The model under review builds one solid part; all positions refer to its coordinate system, in mm. A direction names the side the tool comes from. Give positions to 0.01 mm unless a question says otherwise; leave off trailing zeros. Loops run counter-clockwise (first coordinate to the right, second up) from the corner with the lowest first, then second, coordinate; pieces in that order, holes last. Notation, with made-up numbers: (59, 31.5) -> (82, 31.5) arc R29 ccw to (82, 59.5) -> close; hole circle Ø10 at (-36.5, 3.25). An arc over 180 degrees is marked (long way). Write each question's results on one line, items separated by ' | '. Start each with the question number.
Q1. We need section C-C (z = -59). Write out the cut boundary in (x, y), plus the area to 3 significant figures.
Q2. Wall thickness on L1, parallel to X at y = 4.5, z = -12; L2, parallel to X at y = 8, z = -12; L3, parallel to X at y = 0.75, z = -70: over which ranges is each line inside the solid? List them lowest first. Write a range as [from, to].
Q3. We need section B-B (z = -68). Write out the cut boundary in (x, y).
Q4. We need section A-A (x = 75). Write out the cut boundary in (y, z).
Q5. Mouldability with a two-part tool opening along X and no side actions: class faces 3 (the face through (125, 6, -5)), 4 (the face through (8.242, 8.648, -73.495)), 5 (the face through (64, 12, -41)), 6 (the face through (0, 6, -39)) as released by +X, released by -X, zero draft, split by the parting line, or undercut.
Q6. Insertion check: pin 1 Ø12.5 at (x, z) = (18, -12) entering from +Y; pin 2 Ø5 at (x, z) = (8, -12) entering from +Y. Each pin has a flat end and moves straight along its axis. Give the tip position at first contact, or say it passes through.
Q7. Machinability: for faces 1 (the face through (18, 5.2, -8)), 2 (the face through (65.01, 6.08, -26.58)), which of the approach directions +Z, -Z, +X, -X, +Y, -Y give a long, thin tool a straight path to every point of the face, cutting with its end or side? Answer none if there is none.
Q8. We need section D-D (y = 8.5). Give the number of separate pieces and of enclosed holes in the cut face, plus the area to 3 significant figures.
from build123d import *

# Parameters (mm, degrees)
SKETCH1_W                                            = 130
SKETCH1_H                                            = 80
BOSS_EXTRUDE1_DEPTH                                  = 12
CHAMFER1_SIZE                                        = 10
CBORE_FOR_M6_HEXAGON_SOCKET_HEAD_CAP_SCR_D           = 6.6
CBORE_FOR_M6_HEXAGON_SOCKET_HEAD_CAP_SCR_CBORE_D     = 11
CBORE_FOR_M6_HEXAGON_SOCKET_HEAD_CAP_SCR_CBORE_DEPTH = 6.8
F_6_0MM_DOWEL_HOLE_1_D                               = 6
F_20_0MM_DOWEL_HOLE_1_D                              = 20
SKETCH17_R                                           = 2.5
CUT_EXTRUDE1_DEPTH                                   = 154.114336363


with BuildPart() as part:
    # Sketch1 → Boss-Extrude1 (new body)
    with BuildSketch(Plane(origin=(0, 0, 0), x_dir=(1, 0, 0), z_dir=(0, 1, 0))):
        with Locations((65, 40)):
            Rectangle(SKETCH1_W, SKETCH1_H)
    extrude(amount=BOSS_EXTRUDE1_DEPTH)

    # Chamfer1
    chamfer1_edges = [part.edges().sort_by_distance(p)[0] for p in [
        (130, 6, -80),
        (130, 6, 0),
    ]]
    chamfer(chamfer1_edges, length=CHAMFER1_SIZE)

    # CBORE for M6 Hexagon socket head cap screws1 (through all)
    with Locations(Plane(origin=(8, 12, -68), x_dir=(0, 0, 1), z_dir=(0, 1, 0))):
        with Locations((0, 0), (56, 10)):
            CounterBoreHole(CBORE_FOR_M6_HEXAGON_SOCKET_HEAD_CAP_SCR_D / 2, CBORE_FOR_M6_HEXAGON_SOCKET_HEAD_CAP_SCR_CBORE_D / 2, CBORE_FOR_M6_HEXAGON_SOCKET_HEAD_CAP_SCR_CBORE_DEPTH)

    # Ø6.0mm dowel hole 1 (through all)
    with Locations(Plane(origin=(18, 12, -68), x_dir=(0, 0, 1), z_dir=(0, 1, 0))):
        with Locations((0, 0), (56, -10)):
            Hole(F_6_0MM_DOWEL_HOLE_1_D / 2)

    # Ø20.0mm dowel hole 1 (through all)
    with Locations(Plane(origin=(0, 0, 0), x_dir=(-1, 0, 0), z_dir=(0, -1, 0))):
        with Locations((-75, 52.142135624), (-75, 26.142135624)):
            Hole(F_20_0MM_DOWEL_HOLE_1_D / 2)

    # Sketch17 → Cut-Extrude1 (cut, through all)
    with BuildSketch(Plane(origin=(0, 12, 0), x_dir=(1, 0, 0), z_dir=(0, 1, 0))):
        with Locations(Location((81, 6.142135624, 0), (0, 0, 270))):
            Circle(SKETCH17_R)
        with Locations(Location((69, 72.142135624, 0), (0, 0, 270))):
            Circle(SKETCH17_R)
    extrude(amount=-CUT_EXTRUDE1_DEPTH, mode=Mode.SUBTRACT)


solid = part.part
Output:
1) outline: (0, 0) -> (67.72, 0) -> (67.72, 12) -> (0, 12) -> close; (82.28, 0) -> (130, 0) -> (130, 12) -> (82.28, 12) -> close | area: 1,390 mm2
2) L1: [0, 5], [11, 14.7], [21.3, 130] | L2: [0, 5], [11, 12.5], [23.5, 130] | L3: [0, 5.38], [10.62, 15.76], [20.24, 67.71], [70.29, 130]
3) outline: (0, 0) -> (4.7, 0) -> (4.7, 5.2) -> (2.5, 5.2) -> (2.5, 12) -> (0, 12) -> close; (11.3, 0) -> (15, 0) -> (15, 12) -> (13.5, 12) -> (13.5, 5.2) -> (11.3, 5.2) -> close; (21, 0) -> (130, 0) -> (130, 12) -> (21, 12) -> close
4) outline: (0, -80) -> (12, -80) -> (12, -62.14) -> (0, -62.14) -> close; (0, -42.14) -> (12, -42.14) -> (12, -36.14) -> (0, -36.14) -> close; (0, -16.14) -> (12, -16.14) -> (12, 0) -> (0, 0) -> close
5) face 3: released by +X | face 4: undercut | face 5: zero draft | face 6: released by -X
6) pin 1: y = 12 | pin 2: through
7) face 1: +Y | face 2: +Y, -Y
8) separate pieces: 1 | enclosed holes: 8 | area: 9,390 mm2
